Design review of the part shown in the three views and the two pictorial views. Dimensions are in mm from the part's minimum x, y and z. Give positions to 0.01 mm unless a question says otherwise; leave off trailing zeros. Order: outer loops, then holes, each group sorted by start corner. A loop starts at its lowest first (then second) coordinate and runs counter-clockwise, first axis right, second up. Notation, with made-up numbers: (52.25, 45) - (82.25, 45) arc R16 ccw to (82.25, 71) - close; hole circle Ø5 at (83, 11.5). An arc over 180 degrees is marked (long way). Put each result on its own line as item: value.
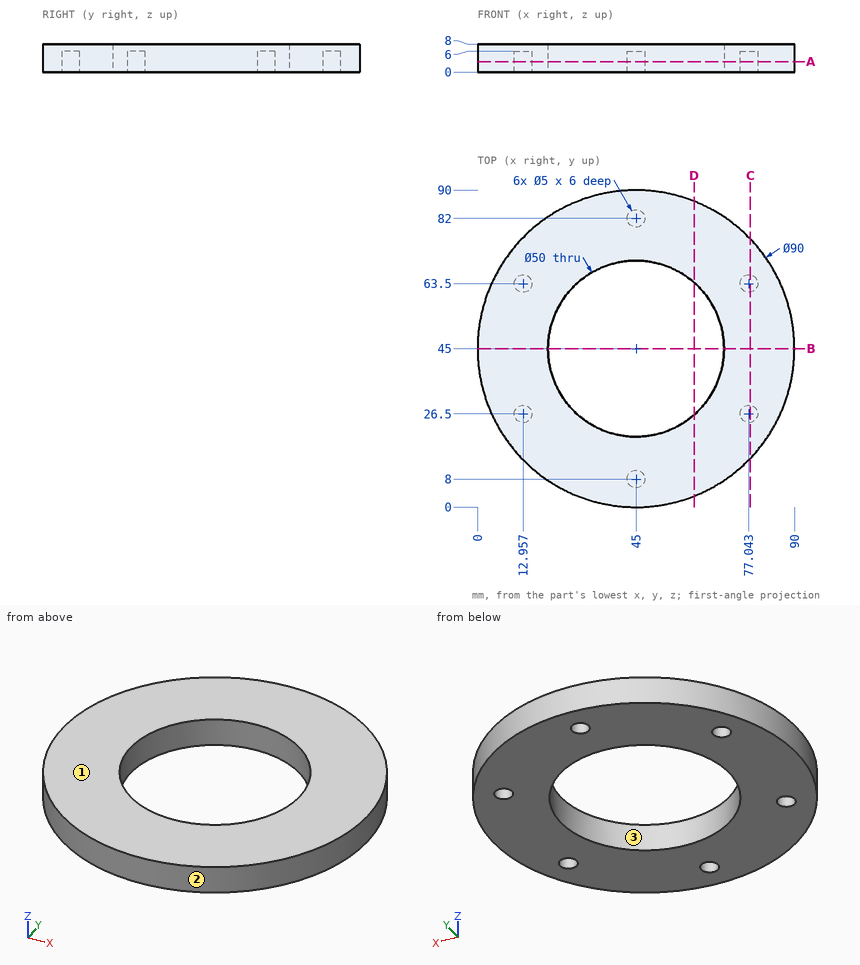
(1) Take a section at D-D, the plane x = 61.5. Write out the cut boundary in (y, z).
The answers:
outline: (3.13, 0) - (26.22, 0) - (26.22, 8) - (3.13, 8) - close; (63.78, 0) - (86.87, 0) - (86.87, 8) - (63.78, 8) - close
(2) Clearance check with flat-ended pins moving along their axes: pin 1 Ø1.5 at (x, y) = (12, 62.5) entering from -Z; pin 2 Ø3 at (y, z) = (19.5, 4.5) entering from -X; pin 3 Ø3 at (x, z) = (43, 3.5) entering from +Y. State where each tip first meets the part, or that it passes through.
The answers:
pin 1: z = 6
pin 2: x = 6.93
pin 3: y = 90
(3) Wall thickness on L1, parallel to Y at x = 45, z = 2.25; L2, parallel to Y at x = 58, z = 1.5; L3, parallel to X at y = 34, z = 3 (3 decimals): over which ranges is each line inside the solid? List them lowest first.
The answers:
L1: 0 to 5.5, 10.5 to 20, 70 to 79.5, 84.5 to 90
L2: 1.92 to 23.65, 66.35 to 88.08
L3: 1.365 to 22.55, 67.45 to 88.635
(4) The part is to be moulded in two halves that separate along Y. For the marked faces 1, 2 and 3, say which applies: pulls with the +Y half, pulls with the -Y half, needs draft (parallel to the pull), parting line crosses it, or undercut.
The answers:
face 1: needs draft
face 2: parting line crosses it
face 3: undercut
(5) Take a section at B-B, the plane y = 45. Write out the cut boundary in (x, z), then the cut area to 3 significant figures.
The answers:
outline: (0, 0) - (20, 0) - (20, 8) - (0, 8) - close; (70, 0) - (90, 0) - (90, 8) - (70, 8) - close
area: 320 mm^2
(6) Take a section at C-C, the plane x = 77.5. Write out the cut boundary in (y, z).
The answers:
outline: (13.88, 0) - (24.04, 0) - (24.04, 6) - (28.96, 6) - (28.96, 0) - (61.04, 0) - (61.04, 6) - (65.96, 6) - (65.96, 0) - (76.12, 0) - (76.12, 8) - (13.88, 8) - close
(7) Take a section at A-A, the plane z = 3. Write out the cut boundary in (x, y).
The answers:
outline: circle Ø90 at (45, 45); hole circle Ø5 at (12.96, 26.5); hole circle Ø5 at (12.96, 63.5); hole circle Ø50 at (45, 45); hole circle Ø5 at (45, 8); hole circle Ø5 at (45, 82); hole circle Ø5 at (77.04, 26.5); hole circle Ø5 at (77.04, 63.5)
